Could you check a few things on this model? Use its own coordinates, in mm. A direction names the side the tool comes from. Give positions to 0.01 mm unless a question says otherwise; leave off trailing zeros. Loops run counter-clockwise (first coordinate to the right, second up) from the corner with the lowest first, then second, coordinate; pieces in that order, holes last. Notation, with made-up numbers: (57, 17.5) - (64, 17.5) arc R18 cw to (64, 27.5) - close; hole circle Ø9 at (67, -14). An arc over 180 degrees is marked (long way). One line per item, written item: value. Start each with the question number.
Q1. I'm going to push flat-ended pins straight in: P1, Ø1, axis at x = 491.5, z = 22.5, coming from the +Y side; P2, Ø10, axis at x = 356.5, z = 104, coming from the -Y side; P3, Ø4.5, axis at x = 596.5, y = -160.5, coming from the +Z side; P4, Ø6, axis at x = 101, z = 150.5, coming from the +Y side. Where does each tip first touch, or does it pass through?
Q2. I want a section at B-B (z = 22). Please give me the cut outline in (x, y).
Q3. I want a section at D-D (x = 423.5). Please give me the cut outline in (y, z).
Q4. If we mould it in two halves opening along Z, with no side actions, what happens to faces 3 (the face through (311.912, -83.577, 89.26)), 4 (the face through (340, -87, 0)), 5 (the face through (222, -51, 178))? For each: released by +Z, released by -Z, zero draft, split by the parting line, or undercut.
Q5. If I drill on line 1 (X direction, y = 98, z = 128); line 2 (Y direction, x = 1, z = 118); line 3 (Y direction, x = 1.5, z = 118), over which ranges is the centre line in solid material (lowest first)? Write a range as from..to.
Q6. I want a section at A-A (z = 118). Please give me the cut outline in (x, y).
Q7. For faces 1 (the face through (2, 65, 87)), 2 (the face through (222, -51, -2)), which set-ups out of +Z, -Z, +X, -X, +Y, -Y let a thin tool reach every point of the face, with its end or its side?
Q8. I want a section at C-C (y = -146). Please give me the cut outline in (x, z), then the cut area to 3 significant figures.
```python
from build123d import *

# Parameters (mm, degrees)
EXTRUDE_THIN1_DEPTH  = 176
EXTRUDE_THIN2_DEPTH  = 2
EXTRUDE_THIN3_DEPTH  = 2
SKETCH4_W            = 2
SKETCH4_H            = 176
BOSS_EXTRUDE1_DEPTH  = 10
CUT_EXTRUDE1_DEPTH   = 2
CUT_EXTRUDE2_DEPTH   = 2
SKETCH7_R            = 7.5
CUT_EXTRUDE3_DEPTH   = 2
LPATTERN3_COUNT      = 2
LPATTERN3_PITCH      = 30
LPATTERN4_COUNT      = 2
LPATTERN4_PITCH      = 70
LPATTERN4_COUNT_DIR2 = 3
LPATTERN4_PITCH_DIR2 = 260
LPATTERN5_COUNT      = 2
LPATTERN5_PITCH      = 70


with BuildPart() as part:
    # Sketch1 → Extrude-Thin1 (new body)
    with BuildSketch(Plane.XY):
        Polygon((632.681416219, -169.526474542), (0, 0), (0, 165), (48, 165), (48, 163), (2, 163), (2, 1.534653976), (633.19905431, -167.59462289), align=None)
    extrude(amount=EXTRUDE_THIN1_DEPTH)

    # Sketch2 → Extrude-Thin2 (add)
    with BuildSketch(Plane.XY.offset(176)):
        Polygon((0, 165), (0, 0), (632.681416219, -169.526474542), (635.787244761, -157.935364627), (12, 9.207923856), (12, 165), align=None)
    extrude(amount=EXTRUDE_THIN2_DEPTH)

    # Sketch3 → Extrude-Thin3 (add)
    with BuildSketch(Plane(origin=(0, 0, 0), x_dir=(-1, 0, 0), z_dir=(0, 0, -1))):
        Polygon((0, 165), (0, 0), (-632.681416219, -169.526474542), (-635.787244761, -157.935364627), (-12, 9.207923856), (-12, 165), align=None)
    extrude(amount=EXTRUDE_THIN3_DEPTH)

    # Sketch4 → Boss-Extrude1 (add)
    with BuildSketch(Plane(origin=(0.51763809, 1.931851653, 0), x_dir=(0.9659258262890673, -0.25881904510252474, 0), z_dir=(0.25881904510252474, 0.9659258262890673, 0))):
        with Locations((654, -88)):
            Rectangle(SKETCH4_W, SKETCH4_H)
    extrude(amount=BOSS_EXTRUDE1_DEPTH)

    # Sketch5 → Cut-Extrude1 (cut)
    with BuildSketch(Plane(origin=(0, 0, 0), x_dir=(0.9659258262890673, -0.2588190451025247, 0), z_dir=(-0.2588190451025247, -0.9659258262890673, 0))):
        with BuildLine():
            Line((611.5, 154), (626.5, 154))
            ThreePointArc((626.5, 154), (632.5, 148), (626.5, 142))
            Line((626.5, 142), (611.5, 142))
            ThreePointArc((611.5, 142), (605.5, 148), (611.5, 154))
        make_face()
    cut_extrude1 = extrude(amount=-CUT_EXTRUDE1_DEPTH, mode=Mode.SUBTRACT)

    # Sketch6 → Cut-Extrude2 (cut)
    with BuildSketch(Plane(origin=(2, 0, 0), x_dir=(0, 0, -1), z_dir=(1, 0, 0))):
        with BuildLine():
            Line((-142, 139.034653976), (-142, 124.034653976))
            ThreePointArc((-142, 124.034653976), (-148, 118.034653976), (-154, 124.034653976))
            Line((-154, 124.034653976), (-154, 139.034653976))
            ThreePointArc((-154, 139.034653976), (-148, 145.034653976), (-142, 139.034653976))
        make_face()
    cut_extrude2 = extrude(amount=-CUT_EXTRUDE2_DEPTH, mode=Mode.SUBTRACT)

    # Sketch7 → Cut-Extrude3 (cut)
    with BuildSketch(Plane.ZY):
        with Locations((88, 85)):
            Circle(SKETCH7_R)
    cut_extrude3 = extrude(amount=-CUT_EXTRUDE3_DEPTH, mode=Mode.SUBTRACT)

    # LPattern3: Cut-Extrude3 ×2
    with Locations(*[(0, 0, i * LPATTERN3_PITCH) for i in range(1, LPATTERN3_COUNT)]):
        add(cut_extrude3, mode=Mode.SUBTRACT)

    # LPattern4: Cut-Extrude1 2 × 3
    with Locations(*[Vector(0, 0, -1) * (i * LPATTERN4_PITCH) + Vector(-0.9659258262890673, 0.2588190451025247, 0) * (j * LPATTERN4_PITCH_DIR2) for i in range(LPATTERN4_COUNT) for j in range(LPATTERN4_COUNT_DIR2) if (i, j) != (0, 0)]):
        add(cut_extrude1, mode=Mode.SUBTRACT)

    # LPattern5: Cut-Extrude2 ×2
    with Locations(*[(0, 0, -i * LPATTERN5_PITCH) for i in range(1, LPATTERN5_COUNT)]):
        add(cut_extrude2, mode=Mode.SUBTRACT)


solid = part.part
```
Worked answers:
1. P1: stops at y = -129.49
1. P2: stops at y = -96.86
1. P3: stops at z = 178
1. P4: passes through
2. outline: (0, 0) - (632.68, -169.53) - (635.79, -157.94) - (633.86, -157.42) - (631.27, -167.08) - (2, 1.53) - (2, 163) - (48, 163) - (48, 165) - (0, 165) - close
3. outline: (-113.48, -2) - (-101.05, -2) - (-101.05, 0) - (-111.41, 0) - (-111.41, 176) - (-101.05, 176) - (-101.05, 178) - (-113.48, 178) - close
4. face 3: zero draft
4. face 4: undercut
4. face 5: released by +Z
5. line 1: x = 0..2
5. line 2: y = -0.27..77.5, 92.5..165
5. line 3: y = -0.4..77.5, 92.5..165
6. outline: (0, 0) - (632.68, -169.53) - (635.79, -157.94) - (633.86, -157.42) - (631.27, -167.08) - (2, 1.53) - (2, 77.5) - (0, 77.5) - close; (0, 92.5) - (2, 92.5) - (2, 163) - (48, 163) - (48, 165) - (0, 165) - close
7. face 1: +X
7. face 2: -Z, +X, -X, +Y, -Y
8. outline: (544.88, -2) - (591.24, -2) - (591.24, 0) - (552.61, 0) - (552.61, 176) - (591.24, 176) - (591.24, 178) - (544.88, 178) - close
8. area: 1,550 mm²
